Verification items for the finished model (mm, model axes). Face numbers are marked on the shaded views. Round coordinates to 2 decimals unless told otherwise and drop trailing zeros. Return JSON: item names as keys, results as strings. Group by question number.
1) Scan lines: L1, parallel to Y at x = -9, z = 9.2 (3 decimals); L2, parallel to Y at x = -9, z = 1.8 (3 decimals); L3, parallel to Y at x = -3, z = 5.5. Record each from-to range of solid material in increasing order.
2) Depth check by flat-ended pin: pin 1 (1.5 mm diameter, centred on x = 33.5, z = 7.5, fed in from +Y); pin 2 (2 mm diameter, centred on x = -7, z = 9, fed in from +Y); pin 3 (2 mm diameter, centred on y = 34, z = 1.5, fed in from -X); pin 4 (3 mm diameter, centred on x = -9, y = 14.5, fed in from +Z). Enter the tip coordinate at first touch or a pass-through.
3) Draft check along X on the marked faces 1, 2 and 3. Enter one of: pulls with the +X half, pulls with the -X half, needs draft (parallel to the pull), parting line crosses it, or undercut.
4) Section check A-A on y = 14.5. State how many separate pieces and enclosed holes the cut face has, plus the area to 3 significant figures.
```python
from build123d import *

# Parameters (mm, degrees)
SKETCH1_W           = 30
SKETCH1_H           = 15
BOSS_EXTRUDE1_DEPTH = 11.9
SKETCH2_W           = 14
SKETCH2_H           = 14
BOSS_EXTRUDE2_DEPTH = 11.9
SKETCH3_R           = 2.525
SKETCH3_R_2         = 1.65
CUT_EXTRUDE2_DEPTH  = 11.9
BOSS_EXTRUDE3_DEPTH = 11.9
SKETCH5_W           = 14
SKETCH5_H           = 4.05
CUT_EXTRUDE3_DEPTH  = 26
FILLET1_R           = 5
FILLET2_R           = 2
SKETCH6_R           = 2.525
CUT_EXTRUDE4_DEPTH  = 3.925


with BuildPart() as part:
    # Sketch1 → Boss-Extrude1 (new body)
    with BuildSketch(Plane.XY):
        Rectangle(SKETCH1_W, SKETCH1_H)
    extrude(amount=BOSS_EXTRUDE1_DEPTH)

    # Sketch2 → Boss-Extrude2 (add)
    with BuildSketch(Plane.XY.offset(11.9)):
        with Locations((-8, 14.5)):
            Rectangle(SKETCH2_W, SKETCH2_H)
    extrude(amount=-BOSS_EXTRUDE2_DEPTH)

    # Sketch3 → Cut-Extrude2 (cut)
    with BuildSketch(Plane.XY.offset(11.9)):
        with Locations((-9, 0.5)):
            Circle(SKETCH3_R)
        with Locations((-9, 14.5)):
            Circle(SKETCH3_R_2)
    extrude(amount=-CUT_EXTRUDE2_DEPTH, mode=Mode.SUBTRACT)

    # Sketch4 → Boss-Extrude3 (add)
    with BuildSketch(Plane.XY.offset(11.9)):
        Polygon((15, -7.5), (106.523733582, 49.690376088), (98.574944619, 62.41109753), (15, 7.5), align=None)
    extrude(amount=-BOSS_EXTRUDE3_DEPTH)

    # Sketch5 → Cut-Extrude3 (cut)
    with BuildSketch(Plane(origin=(0, 7.5, 0), x_dir=(1, 0, 0), z_dir=(0, 1, 0))):
        with Locations((-8, -5.95)):
            Rectangle(SKETCH5_W, SKETCH5_H)
    extrude(amount=CUT_EXTRUDE3_DEPTH, mode=Mode.SUBTRACT)

    # Fillet1
    fillet1_edges = [part.edges().sort_by_distance(p)[0] for p in [
        (-15, 21.5, 1.9625),
        (-1, 21.5, 1.9625),
        (-1, 7.5, 1.9625),
        (98.574944619, 62.41109753, 5.95),
        (106.523733582, 49.690376088, 5.95),
        (-1, 21.5, 9.9375),
        (-1, 7.5, 9.9375),
        (-15, 21.5, 9.9375),
        (15, -7.5, 5.95),
        (-15, -7.5, 5.95),
        (15, 7.5, 5.95),
    ]]
    fillet(fillet1_edges, radius=FILLET1_R)

    # Fillet2
    fillet2_edges = [part.edges().sort_by_distance(p)[0] for p in [
        (14.937271043, 7.709711065, 0),
        (14.937271043, 7.709711065, 11.9),
        (0.464466094, 8.964466094, 11.9),
        (0.464466094, 8.964466094, 0),
        (102.579887045, 56.001849878, 0),
        (102.579887045, 56.001849878, 11.9),
        (1.783136536, -7.5, 11.9),
        (59.249681247, 20.150269643, 11.9),
        (55.274895994, 33.961743433, 11.9),
        (8.75219782, 7.5, 11.9),
        (-1, 14.5, 11.9),
        (-8, 21.5, 11.9),
        (-15, 7, 11.9),
        (-13.535533906, 20.035533906, 11.9),
        (-2.464466094, 20.035533906, 11.9),
        (-13.535533906, -6.035533906, 11.9),
        (14.94445985, -7.30630848, 11.9),
        (104.505747104, 50.156264976, 11.9),
        (98.114553442, 60.307839752, 11.9),
        (55.274895994, 33.961743433, 0),
        (8.75219782, 7.5, 0),
        (59.249681247, 20.150269643, 0),
        (1.783136536, -7.5, 0),
        (-15, 7, 0),
        (-8, 21.5, 0),
        (-1, 14.5, 0),
        (-13.535533906, 20.035533906, 0),
        (-2.464466094, 20.035533906, 0),
        (-13.535533906, -6.035533906, 0),
        (14.94445985, -7.30630848, 0),
        (104.505747104, 50.156264976, 0),
        (98.114553442, 60.307839752, 0),
    ]]
    fillet(fillet2_edges, radius=FILLET2_R)

    # Sketch6 → Cut-Extrude4 (cut)
    with BuildSketch(Plane.XY.offset(11.9)):
        with Locations((-9, 14.5)):
            Circle(SKETCH6_R)
    extrude(amount=-CUT_EXTRUDE4_DEPTH, mode=Mode.SUBTRACT)


solid = part.part
```
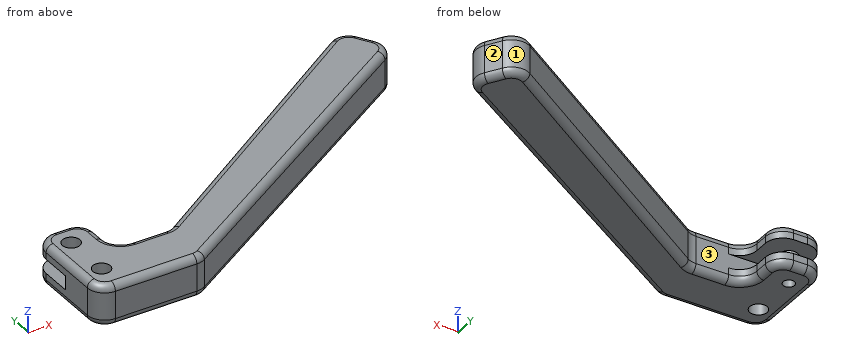
Check result:
{
 "1": {"L1": "-7.5 to -2.025, 3.025 to 11.975, 17.025 to 21.5", "L2": "-7.49 to -2.025, 3.025 to 12.85, 16.15 to 21.49", "L3": "-7.5 to 7.5"},
 "2": {"pin 1": "y = 20.15", "pin 2": "y = 21.5", "pin 3": "x = 53.88", "pin 4": "through"},
 "3": {"face 1": "parting line crosses it", "face 2": "pulls with the +X half", "face 3": "undercut"},
 "4": {"separate pieces": "5", "enclosed holes": "0", "area": "360 mm^2"}
}
